```python
from build123d import *

# Parameters (mm, degrees)
SKETCH1_R           = 5
SKETCH1_W           = 8.3
SKETCH1_H           = 28
BOSS_EXTRUDE2_DEPTH = 8.3
SKETCH2_R           = 3
BOSS_EXTRUDE4_DEPTH = 8.3


with BuildPart() as part:
    # Sketch1 → Boss-Extrude2 (new body)
    # profile 1 of 2: a face of its own
    with BuildSketch(Plane.XY):
        with BuildLine():
            Line((-29.9, 14), (0, 14))
            Line((0, 14), (0, -14))
            Line((0, -14), (-29.9, -14))
            ThreePointArc((-29.9, -14), (-43.9, 0), (-29.9, 14))
        make_face()
        with Locations(Location((-29.9, 0, 0), (0, 0, 180))):
            Circle(SKETCH1_R, mode=Mode.SUBTRACT)
    # profile 2 of 2: a face of its own
    with BuildSketch(Plane.XY):
        with Locations((4.15, 0)):
            Rectangle(SKETCH1_W, SKETCH1_H)
    extrude(amount=BOSS_EXTRUDE2_DEPTH)

    # Sketch2 → Boss-Extrude4 (add)
    with BuildSketch(Plane.XY.offset(8.3)):
        with BuildLine():
            Line((0, 14), (0, -14))
            Line((0, -14), (18.211120602, -14))
            Line((18.211120602, -14), (56.77473573, -8.923003752))
            ThreePointArc((56.77473573, -8.923003752), (64.6, 0), (56.77473573, 8.923003752))
            Line((56.77473573, 8.923003752), (18.211120602, 14))
            Line((18.211120602, 14), (0, 14))
        make_face()
        with Locations(Location((55.6, 0, 0), (0, 0, 180))):
            Circle(SKETCH2_R, mode=Mode.SUBTRACT)
    extrude(amount=BOSS_EXTRUDE4_DEPTH)


solid = part.part
```
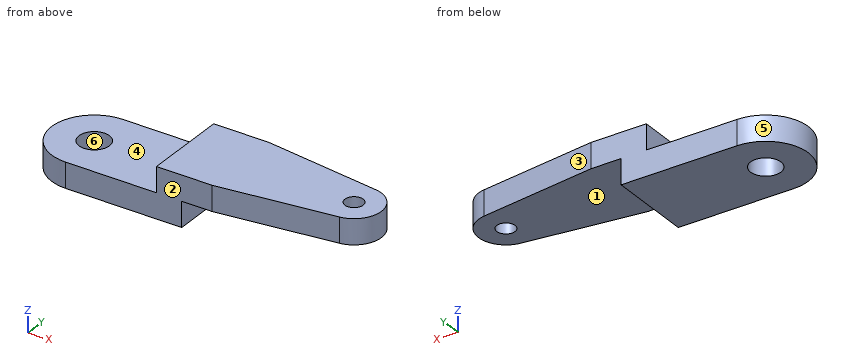
The listing builds one solid part. Answer for the finished solid, in the listing's coordinates (mm). Face numbers are marked on the shaded views. A direction names the side the tool comes from. Coordinates: 2 decimals unless noted, no trailing zeros. Write each loop counter-clockwise with the first axis right and the second up, starting at its lowest first coordinate (ties: lowest second). Pieces come first, ordered by that corner, then holes. Notation, with made-up numbers: M 52,68.25 L 65,68.25 A23 ccw 65,107.25 Z; hole C -25,22 d9. An arc over 180 degrees is marked long. Use a Markdown table: item, result. Add a question column.
1. For a pull along Y with two mould halves and no side action, classify the marked faces 3, 4, 5 and 6 as +Y half, -Y half, draft (parallel to the pull), parting line (faces both ways), or undercut.
2. Section D-D (y = 4) is taken. Give the vertices of the cut face in (x, z), plus the area to 3 significant figures.
3. Section B-B (z = 14.25) is taken. Give the vertices of the cut face in (x, y), plus the area to 3 significant figures.
4. Which of the six approach directions +Z, -Z, +X, -X, +Y, -Y give full straight-line access (tool end or side, diameter ignored) to the marked faces 1 and 2?
5. Given P1, Ø4, axis at x = -14, z = 8.5, coming from the +Y side; P2, Ø2, axis at y = -8.5, z = 3.5, coming from the -X side; P3, Ø8, axis at y = -7, z = 4, coming from the +X side; P4, Ø2, axis at x = 35.5, z = 10.5, coming from the +Y side, each flat-ended and moving along its own axis, determine where each tip first touches the part or whether it passes through.
6. Section A-A (y = 0) is taken. Give the vertices of the cut face in (x, z), plus the area to 3 significant figures.
7. Straight lines are drawn through the part: line 1 along Y through (x, z) = (-29.9, 3.5); line 2 along Z through (x, y) = (-18.5, 4.25); line 3 along Z through (x, y) = (21.5, 7.75). For each, find the intervals that lie inside material, in ascending order. Write a range as [from, to].
8. Section C-C (x = 55.6) is taken. Give the vertices of the cut face in (y, z).
Data:
| question | item | result |
|---|---|---|
| 1 | face 3 | +Y half |
| 1 | face 4 | draft |
| 1 | face 5 | parting line |
| 1 | face 6 | undercut |
| 2 | outline | M -43.32,0 L -32.9,0 L -32.9,8.3 L -43.32,8.3 Z; M -26.9,0 L 8.3,0 L 8.3,8.3 L 63.66,8.3 L 63.66,16.6 L 0,16.6 L 0,8.3 L -26.9,8.3 Z |
| 2 | area | 907 mm2 |
| 3 | outline | M 0,-14 L 18.21,-14 L 56.77,-8.92 A9 ccw 56.77,8.92 L 18.21,14 L 0,14 Z; hole C 55.6,0 d6 |
| 3 | area | 1,470 mm2 |
| 4 | face 1 | -Z, +X, +Y, -Y |
| 4 | face 2 | +Z, -Z, +X, -X, -Y |
| 5 | P1 | stops at y = 14 |
| 5 | P2 | stops at x = -41.72 |
| 5 | P3 | stops at x = 8.3 |
| 5 | P4 | stops at y = 11.86 |
| 6 | outline | M -43.9,0 L -34.9,0 L -34.9,8.3 L -43.9,8.3 Z; M -24.9,0 L 8.3,0 L 8.3,8.3 L 52.6,8.3 L 52.6,16.6 L 0,16.6 L 0,8.3 L -24.9,8.3 Z; M 58.6,8.3 L 64.6,8.3 L 64.6,16.6 L 58.6,16.6 Z |
| 6 | area | 837 mm2 |
| 7 | line 1 | y = [-14, -5], [5, 14] |
| 7 | line 2 | z = [0, 8.3] |
| 7 | line 3 | z = [8.3, 16.6] |
| 8 | outline | M -9.08,8.3 L -3,8.3 L -3,16.6 L -9.08,16.6 Z; M 3,8.3 L 9.08,8.3 L 9.08,16.6 L 3,16.6 Z |
